The drawing under review shows one solid part. Ordinate dimensions are in mm from its lowest x, y, z. Coordinates: 2 decimals unless noted, no trailing zeros. Order: outer loops, then holes, each group sorted by start corner. A loop starts at its lowest first (then second) coordinate and runs counter-clockwise, first axis right, second up.
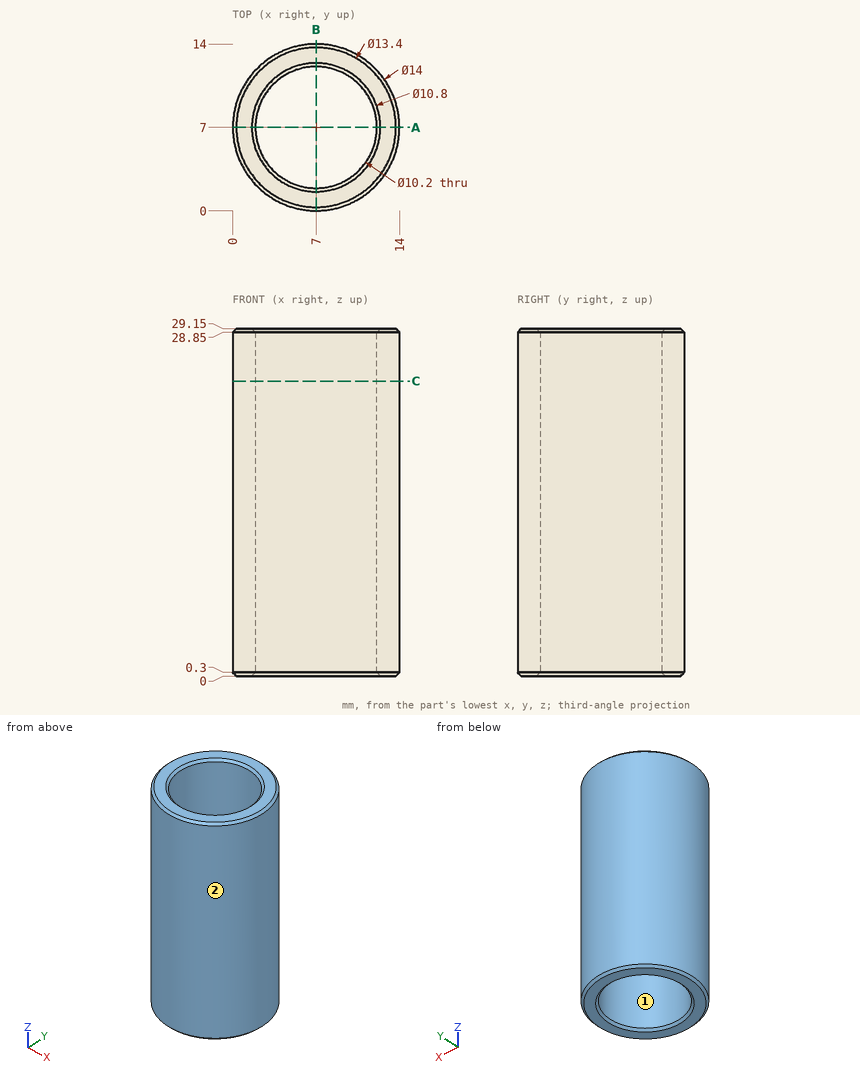
1. Take a section at C-C, the plane z = 24.75. Give the boundary of the cut face in (x, y).
Answer below:
outline: circle Ø14 at (7, 7); hole circle Ø10.2 at (7, 7)
2. The part is to be moulded in two halves that separate along Y. For the marked faces 1 and 2, say which applies: +Y half, -Y half, draft (parallel to the pull), parting line (faces both ways), or undercut.
Answer below:
face 1: undercut
face 2: parting line
3. Clearance check with flat-ended pins moving along their axes: pin 1 Ø1 at (y, z) = (5.5, 19.5) entering from -X; pin 2 Ø2 at (x, z) = (2.5, 11.5) entering from -Y; pin 3 Ø5 at (x, z) = (12, 10.5) entering from -Y. State where each tip first meets the part, or that it passes through.
Answer below:
pin 1: stops at x = 0.07
pin 2: stops at y = 0.94
pin 3: stops at y = 0.46
4. Take a section at A-A, the plane y = 7. Give the boundary of the cut face in (x, z), plus the area to 3 significant figures.
Answer below:
outline: (0, 0.3) - (0.3, 0) - (1.6, 0) - (1.9, 0.3) - (1.9, 28.85) - (1.6, 29.15) - (0.3, 29.15) - (0, 28.85) - close; (12.1, 0.3) - (12.4, 0) - (13.7, 0) - (14, 0.3) - (14, 28.85) - (13.7, 29.15) - (12.4, 29.15) - (12.1, 28.85) - close
area: 110 mm2
5. To check wall thickness, follow L1, parallel to Y at x = 7, z = 21.75; L2, parallel to X at y = 3.5, z = 13.75; L3, parallel to X at y = 10.25, z = 15.5. State the ranges of each line that lie inside material, in increasing order.
Answer below:
L1: y = 0 to 1.9, 12.1 to 14
L2: x = 0.94 to 3.29, 10.71 to 13.06
L3: x = 0.8 to 3.07, 10.93 to 13.2
